For this review, take the finished solid that the model builds, in its own axes (mm). Face numbers are marked on the shaded views. Coordinates: 2 decimals unless noted, no trailing zeros. Order: outer loops, then holes, each group sorted by start corner. A loop starts at its lowest first (then second) coordinate and runs counter-clockwise, first axis right, second up.
from build123d import *

# Parameters (mm, degrees)
SKETCH1_W           = 42.7
SKETCH1_H           = 55.3
BOSS_EXTRUDE1_DEPTH = 37.7
CUT_EXTRUDE1_REACH  = 65.317
SKETCH4_W           = 10
SKETCH4_H           = 5
BOSS_EXTRUDE2_DEPTH = 4


with BuildPart() as part:
    # Sketch1 → Boss-Extrude1 (new body)
    with BuildSketch(Plane(origin=(0, 0, 0), x_dir=(1, 0, 0), z_dir=(0, 1, 0))):
        Rectangle(SKETCH1_W, SKETCH1_H)
    extrude(amount=BOSS_EXTRUDE1_DEPTH)

    # Sketch3 → Cut-Extrude1 (cut, up to next)
    with BuildSketch(Plane(origin=(21.35, 0, 0), x_dir=(0, 0, -1), z_dir=(1, 0, 0)), mode=Mode.PRIVATE) as cut_extrude1_sk1:
        Polygon((-15.25, 0), (-15.25, 1.8), (-16.95, 1.8), (-16.95, 3), (18.399583247, 3), (18.399583247, 1.8), (16.95, 1.8), (16.95, 0), align=None)
    cut_extrude1_tool1 = extrude(cut_extrude1_sk1.sketch, amount=-CUT_EXTRUDE1_REACH, mode=Mode.PRIVATE) & part.part
    add(cut_extrude1_tool1.solids().sort_by_distance((21.35, 1.533887, -0.797088))[0], mode=Mode.SUBTRACT)

    # Sketch4 → Boss-Extrude2 (add)
    with BuildSketch(Plane.XZ):
        with Locations((16.35, -30.15)):
            Rectangle(SKETCH4_W, SKETCH4_H)
    extrude(amount=-BOSS_EXTRUDE2_DEPTH)


solid = part.part
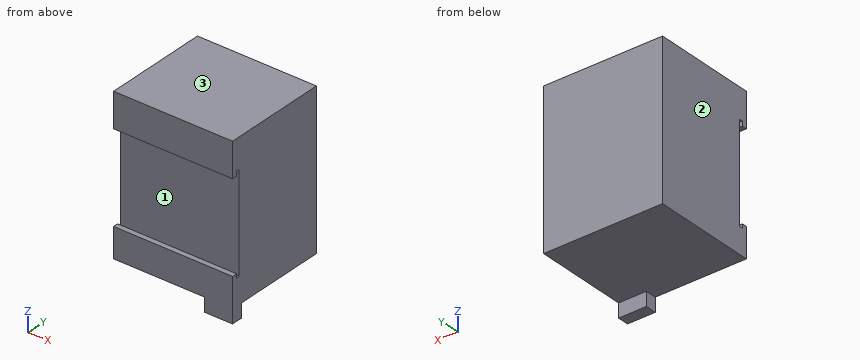
1. To check wall thickness, follow L1, parallel to Y at x = 9.5, z = -4; L2, parallel to Y at x = -15, z = -17; L3, parallel to Z at x = -16.5, y = 18. State the ranges of each line that lie inside material, in increasing order.
Answer below:
L1: y = 3 to 37.7
L2: y = 0 to 1.8, 3 to 37.7
L3: z = -27.65 to 27.65
2. The part is to be moulded in two halves that separate along Z. For the marked faces 1, 2 and 3, say which applies: +Z half, -Z half, draft (parallel to the pull), parting line (faces both ways), or undercut.
Answer below:
face 1: undercut
face 2: draft
face 3: +Z half
3. Clearance check with flat-ended pins moving along their axes: pin 1 Ø1.5 at (x, y) = (17, 5) entering from -Z; pin 2 Ø4 at (x, z) = (17, -29.5) entering from +Y; pin 3 Ø1 at (x, z) = (-1.5, -2) entering from -Y; pin 4 Ø3 at (y, z) = (1, -30) entering from -X. State where each tip first meets the part, or that it passes through.
Answer below:
pin 1: stops at z = -27.65
pin 2: stops at y = 37.7
pin 3: stops at y = 3
pin 4: stops at x = 11.35
4. Take a section at C-C, the plane y = 26. Give the boundary of the cut face in (x, z), plus the area to 3 significant figures.
Answer below:
outline: (-21.35, -27.65) - (21.35, -27.65) - (21.35, 27.65) - (-21.35, 27.65) - close
area: 2,360 mm2
5. Take a section at B-B, the plane z = 7. Give the boundary of the cut face in (x, y).
Answer below:
outline: (-21.35, 3) - (21.35, 3) - (21.35, 37.7) - (-21.35, 37.7) - close
6. Take a section at A-A, the plane x = 9. Give the boundary of the cut face in (y, z), plus the area to 3 significant figures.
Answer below:
outline: (0, -27.65) - (37.7, -27.65) - (37.7, 27.65) - (0, 27.65) - (0, 15.25) - (1.8, 15.25) - (1.8, 16.95) - (3, 16.95) - (3, -18.4) - (1.8, -18.4) - (1.8, -16.95) - (0, -16.95) - close
area: 1,980 mm2
7. Take a section at D-D, the plane x = 15. Give the boundary of the cut face in (y, z), plus the area to 3 significant figures.
Answer below:
outline: (0, -32.65) - (4, -32.65) - (4, -27.65) - (37.7, -27.65) - (37.7, 27.65) - (0, 27.65) - (0, 15.25) - (1.8, 15.25) - (1.8, 16.95) - (3, 16.95) - (3, -18.4) - (1.8, -18.4) - (1.8, -16.95) - (0, -16.95) - close
area: 2,000 mm2
